The listing builds one solid part. Answer for the finished solid, in the listing's coordinates (mm). Face numbers are marked on the shaded views. Coordinates: 2 decimals unless noted, no trailing zeros. Order: outer loops, then holes, each group sorted by start corner. A loop starts at its lowest first (then second) coordinate and runs counter-clockwise, first axis right, second up. Notation, with made-up numbers: (-23.5, 77) - (-15.5, 77) arc R7 cw to (-15.5, 81) - close; hole circle Ø10 at (17.25, 41.25). An arc over 180 degrees is marked (long way). Use a Markdown table: item, result. Add a question column.
Item 1: The part is cut by section C-C, the plane y = 4. Give the vertices of the cut face in (x, z).
Item 2: The part is cut by section A-A, the plane z = 0. Give the vertices of the cut face in (x, y).
Item 3: Flat-ended cylindrical pins translate along their axes: P1, Ø1.5, axis at x = -14.5, y = 6.5, coming from the -Z side; P2, Ø7, axis at x = 0, z = 0, coming from the -Y side; P3, Ø4, axis at y = 6, z = -15, coming from the -X side; P4, Ø1.5, axis at x = 11.5, y = 4.5, coming from the +Z side. Find the tip coordinate at first contact, or state that the pin passes through.
Item 4: Find the intervals of material crossed by line 1 along X through (y, z) = (4.7, 0); line 2 along X through (y, z) = (2, 2); line 3 along X through (y, z) = (4.5, 21), in increasing order.
Item 5: The part is cut by section B-B, the plane x = 0. Give the vertices of the cut face in (y, z), then the cut area to 3 significant figures.
Item 6: The mould has two halves that part along X. Classify the marked faces 1, 2 and 3: released by +X, released by -X, zero draft, split by the parting line, or undercut.
from build123d import *


with BuildPart() as part:
    # 草图1 → 旋转1 (revolve)
    with BuildSketch(Plane.XY, mode=Mode.PRIVATE) as revolve_1_sk:
        Polygon((24, 8), (5.5, 8), (4.5, 7), (4.5, 1), (5.5, 0), (24, 0), (25, 1), (25, 7), align=None)
    revolve(revolve_1_sk.sketch.rotate(Axis((0, 8, 0), (0, -1, 0)), 270), axis=Axis((0, 8, 0), (0, -1, 0)))


solid = part.part
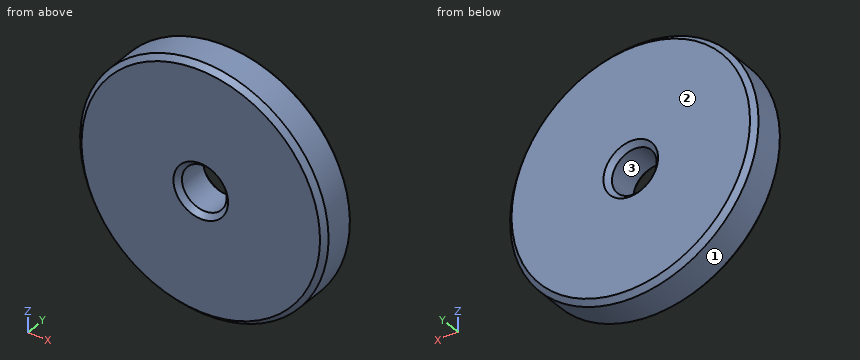
Solution:
| question | item | result |
|---|---|---|
| 1 | outline | circle Ø50 at (0, 0); hole circle Ø9 at (0, 0) |
| 2 | outline | (-25, 1) - (-24, 0) - (-5.5, 0) - (-4.5, 1) - (-4.5, 7) - (-5.5, 8) - (-24, 8) - (-25, 7) - close; (4.5, 1) - (5.5, 0) - (24, 0) - (25, 1) - (25, 7) - (24, 8) - (5.5, 8) - (4.5, 7) - close |
| 3 | P1 | stops at z = -20.88 |
| 3 | P2 | passes through |
| 3 | P3 | stops at x = -21.35 |
| 3 | P4 | stops at z = 22.57 |
| 4 | line 1 | x = -25 to -4.5, 4.5 to 25 |
| 4 | line 2 | x = -24.92 to -4.03, 4.03 to 24.92 |
| 4 | line 3 | x = -13.56 to 13.56 |
| 5 | outline | (0, -24) - (1, -25) - (7, -25) - (8, -24) - (8, -5.5) - (7, -4.5) - (1, -4.5) - (0, -5.5) - close; (0, 5.5) - (1, 4.5) - (7, 4.5) - (8, 5.5) - (8, 24) - (7, 25) - (1, 25) - (0, 24) - close |
| 5 | area | 324 mm2 |
| 6 | face 1 | split by the parting line |
| 6 | face 2 | zero draft |
| 6 | face 3 | undercut |
